Could you check a few things on this model? Use its own coordinates, in mm. Give positions to 0.01 mm unless a question says otherwise; leave off trailing zeros. Loops run counter-clockwise (first coordinate to the right, second up) from the corner with the lowest first, then second, coordinate; pieces in that order, holes last. Notation, with made-up numbers: (0, 69) -> (33, 69) arc R27 ccw to (33, 100) -> close; hole circle Ø7 at (24.25, -39). An arc over 180 degrees is marked (long way). Write item = value, one per line. Start each with the question number.
1) I want a section at B-B (z = 1.5). List the corners of the cut face in (x, y) for me.
2) If we mould it in two halves opening along Y, with no side actions, what happens to faces 1 (the face through (-0.46, 23.47, 5.07)), 2 (the face through (0, -30, 5)), 3 (the face through (12.5, -3, 5)), 4 (the face through (-0.46, -21.53, 5.07))? For each: +Y half, -Y half, draft (parallel to the pull), parting line (faces both ways), or undercut.
3) I want a section at D-D (x = 8.5). List the corners of the cut face in (y, z) for me.
4) I need wall thicknesses on probe 1 along Y at (x, z) = (0, 3.5); probe 2 along X at (y, z) = (-22, 6.5); probe 3 along X at (y, z) = (-23, 4.5). Which ranges of each line are inside material? Lowest first, please. Write a range as from..to.
5) I want a section at A-A (x = 0). List the corners of the cut face in (y, z) for me.
6) I want a section at C-C (y = 20). List the corners of the cut face in (x, z) for me, and give its area (3 significant figures).
from build123d import *

# Parameters (mm, degrees)
SKETCH1_W           = 25
SKETCH1_H           = 60
BOSS_EXTRUDE1_DEPTH = 10
SKETCH2_R           = 3.5
CUT_EXTRUDE1_DEPTH  = 10
CHAMFER1_SIZE       = 5


with BuildPart() as part:
    # Sketch1 → Boss-Extrude1 (new body)
    with BuildSketch(Plane.XY):
        Rectangle(SKETCH1_W, SKETCH1_H)
    extrude(amount=BOSS_EXTRUDE1_DEPTH)

    # Sketch2 → Cut-Extrude1 (cut)
    with BuildSketch(Plane.XY.offset(10)):
        with Locations((0, 20)):
            Circle(SKETCH2_R)
        with Locations((0, -25)):
            Circle(SKETCH2_R)
    extrude(amount=-CUT_EXTRUDE1_DEPTH, mode=Mode.SUBTRACT)

    # Chamfer1
    chamfer1_edges = [part.edges().sort_by_distance(p)[0] for p in [
        (-12.5, 30, 5),
        (12.5, 30, 5),
    ]]
    chamfer(chamfer1_edges, length=CHAMFER1_SIZE)


solid = part.part
Answer list:
q1.outline = (-12.5, -30) -> (12.5, -30) -> (12.5, 25) -> (7.5, 30) -> (-7.5, 30) -> (-12.5, 25) -> close; hole circle Ø7 at (0, -25); hole circle Ø7 at (0, 20)
q2.face_1 = undercut
q2.face_2 = -Y half
q2.face_3 = draft
q2.face_4 = undercut
q3.outline = (-30, 0) -> (29, 0) -> (29, 10) -> (-30, 10) -> close
q4.probe_1 = -30..-28.5, -21.5..16.5, 23.5..30
q4.probe_2 = -12.5..-1.8, 1.8..12.5
q4.probe_3 = -12.5..-2.87, 2.87..12.5
q5.outline = (-30, 0) -> (-28.5, 0) -> (-28.5, 10) -> (-30, 10) -> close; (-21.5, 0) -> (16.5, 0) -> (16.5, 10) -> (-21.5, 10) -> close; (23.5, 0) -> (30, 0) -> (30, 10) -> (23.5, 10) -> close
q6.outline = (-12.5, 0) -> (-3.5, 0) -> (-3.5, 10) -> (-12.5, 10) -> close; (3.5, 0) -> (12.5, 0) -> (12.5, 10) -> (3.5, 10) -> close
q6.area = 180 mm^2
